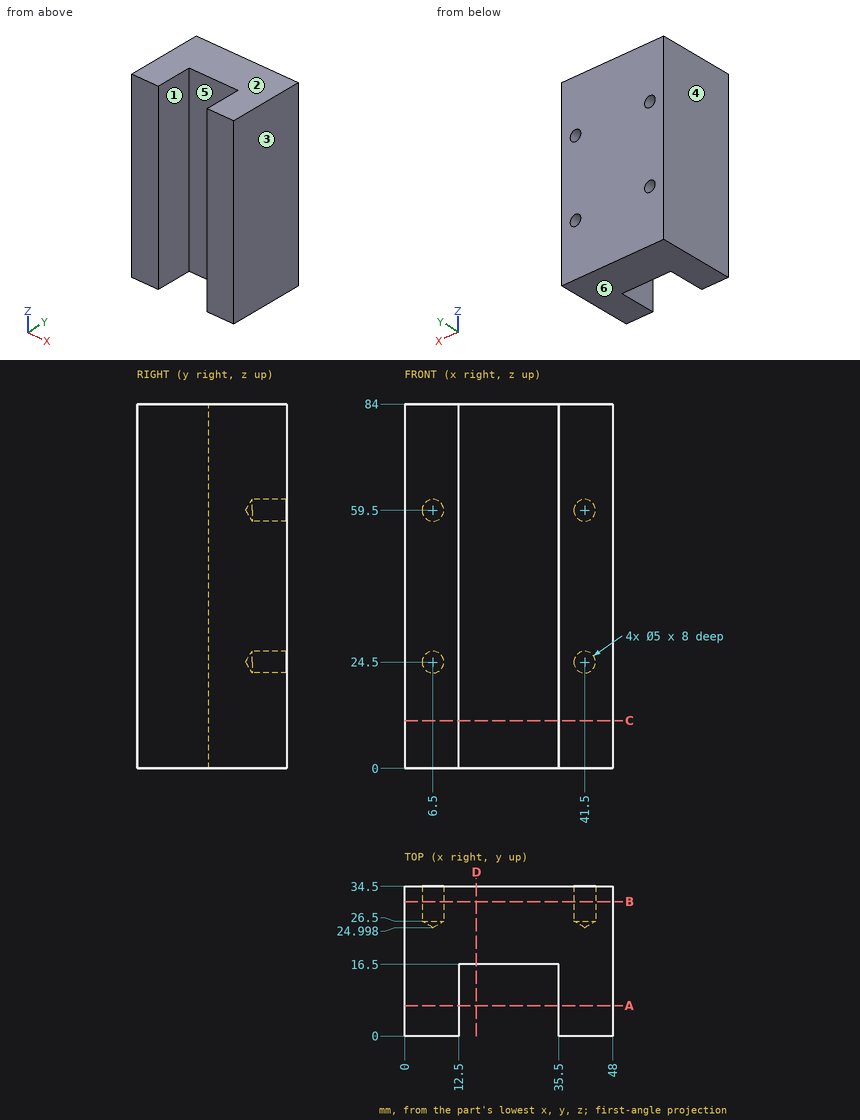
Could you check a few things on this drawing? It's one solid part, dimensions in mm from its lowest x, y, z. A direction names the side the tool comes from. Coordinates: 2 decimals unless noted, no trailing zeros. Loops run counter-clockwise (first coordinate to the right, second up) from the corner with the lowest first, then second, coordinate; pieces in that order, holes last.
1. For P1, Ø4, axis at x = 41.5, z = 24.5, coming from the +Y side; P2, Ø18.5, axis at x = 23.5, z = 31.5, coming from the -Y side; P3, Ø4.5, axis at x = 6.5, z = 24.5, coming from the +Y side, each with a flat end and sliding along its axis, tell me the tip position at first contact or that it passes through.
2. Imagine slicing it at D-D (x = 16.5). Please give me the cut outline in (y, z).
3. I need wall thicknesses on L1, parallel to Z at x = 41.5, y = 29; L2, parallel to X at y = 30.75, z = 24.5; L3, parallel to X at y = 3, z = 74.5. Which ranges of each line are inside material? Lowest first, please.
4. Imagine slicing it at A-A (y = 7). Please give me the cut outline in (x, z).
5. For the marked faces 5 and 6, which set-ups out of +Z, -Z, +X, -X, +Y, -Y let a thin tool reach every point of the face, with its end or its side?
6. Imagine slicing it at B-B (y = 31). Please give me the cut outline in (x, z).
7. Imagine slicing it at C-C (z = 11). Please give me the cut outline in (x, y).
8. We'd pull the mould along X, two halves only. Please class the marked faces 1, 2, 3 and 4: released by +X, released by -X, zero draft, split by the parting line, or undercut.
Computed values:
1. P1: stops at y = 26.2
1. P2: stops at y = 16.5
1. P3: stops at y = 26.35
2. outline: (16.5, 0) - (34.5, 0) - (34.5, 84) - (16.5, 84) - close
3. L1: z = 0 to 22, 27 to 57, 62 to 84
3. L2: x = 0 to 4, 9 to 39, 44 to 48
3. L3: x = 0 to 12.5, 35.5 to 48
4. outline: (0, 0) - (12.5, 0) - (12.5, 84) - (0, 84) - close; (35.5, 0) - (48, 0) - (48, 84) - (35.5, 84) - close
5. face 5: +Z, -Z, -Y
5. face 6: -Z, +X, -X, +Y, -Y
6. outline: (0, 0) - (48, 0) - (48, 84) - (0, 84) - close; hole circle Ø5 at (6.5, 24.5); hole circle Ø5 at (6.5, 59.5); hole circle Ø5 at (41.5, 24.5); hole circle Ø5 at (41.5, 59.5)
7. outline: (0, 0) - (12.5, 0) - (12.5, 16.5) - (35.5, 16.5) - (35.5, 0) - (48, 0) - (48, 34.5) - (0, 34.5) - close
8. face 1: undercut
8. face 2: zero draft
8. face 3: released by +X
8. face 4: released by -X
